Geometry: see drawing. Coordinates: mm, zero at the bounding-box minimum. A direction names the side the tool comes from. Give positions to 0.01 mm unless a question says otherwise; leave off trailing zeros. Order: outer loops, then holes, each group sorted by start corner. A loop starts at its lowest first (then second) coordinate and runs counter-clockwise, first axis right, second up. Notation, with made-up numbers: (83, 3) - (90, 3) arc R21 ccw to (90, 32) - close; hole circle Ø10 at (-36.75, 83.5). An arc over 180 degrees is marked (long way). One line per item, written item: value.
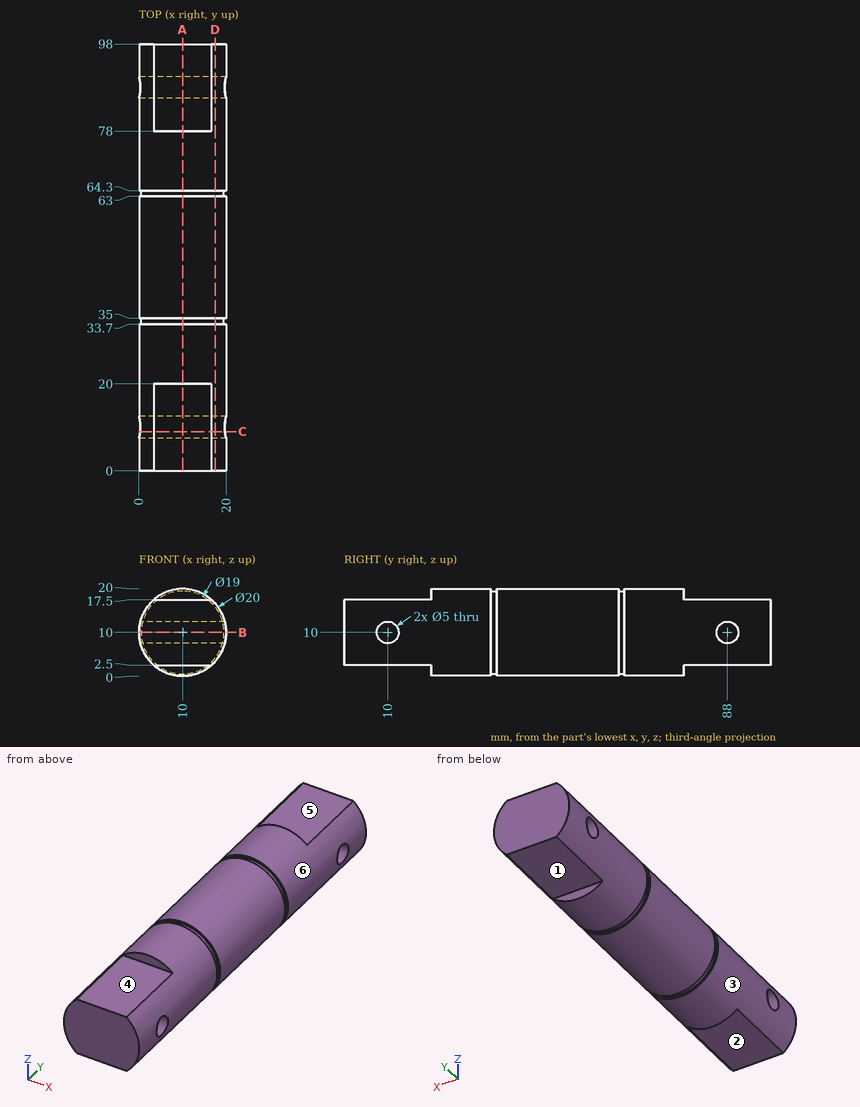
1) Section D-D, the plane x = 17.5. Return loops of the section in (y, z), then the cut area to 3 significant figures.
Answers below:
outline: (0, 3.39) - (33.7, 3.39) - (33.7, 4.17) - (35, 4.17) - (35, 3.39) - (63, 3.39) - (63, 4.17) - (64.3, 4.17) - (64.3, 3.39) - (98, 3.39) - (98, 16.61) - (64.3, 16.61) - (64.3, 15.83) - (63, 15.83) - (63, 16.61) - (35, 16.61) - (35, 15.83) - (33.7, 15.83) - (33.7, 16.61) - (0, 16.61) - close; hole circle Ø5 at (10, 10); hole circle Ø5 at (88, 10)
area: 1,250 mm^2
2) Section B-B, the plane z = 10. Return loops of the section in (x, y).
Answers below:
outline: (0, 0) - (20, 0) - (20, 7.5) - (0, 7.5) - close; (0, 12.5) - (20, 12.5) - (20, 33.7) - (19.5, 33.7) - (19.5, 35) - (20, 35) - (20, 63) - (19.5, 63) - (19.5, 64.3) - (20, 64.3) - (20, 85.5) - (0, 85.5) - (0, 64.3) - (0.5, 64.3) - (0.5, 63) - (0, 63) - (0, 35) - (0.5, 35) - (0.5, 33.7) - (0, 33.7) - close; (0, 90.5) - (20, 90.5) - (20, 98) - (0, 98) - close
3) First-contact query: pin 1 (0.8 mm diameter, centred on x = 11.5, z = 0.5, fed in from -Y); pin 2 (3 mm diameter, centred on x = 5.5, y = 29, fed in from -Z); pin 3 (0.8 mm diameter, centred on x = 7.5, z = 0.5, fed in from +Y). Flat tips, straight axial feed; report the tip coordinate or a pass-through.
Answers below:
pin 1: y = 20
pin 2: z = 0.46
pin 3: y = 78
4) Mould query, pull axis X, two halves, no side actions, for the marked faces 5 and 6. Classes: released by +X, released by -X, zero draft, split by the parting line, or undercut.
Answers below:
face 5: zero draft
face 6: split by the parting line
5) Set-up query: the marked faces 1, 2, 3 and 4. Return all of +Z, -Z, +X, -X, +Y, -Y with unobstructed straight access to the full face (end or side cutting, diameter ignored); none if empty.
Answers below:
face 1: -Z, +X, -X, +Y
face 2: -Z, +X, -X, -Y
face 3: +Y, -Y
face 4: +Z, +X, -X, -Y
6) Section C-C, the plane y = 9. Return loops of the section in (x, z).
Answers below:
outline: (0.27, 7.71) arc R10 ccw to (3.39, 2.5) - (16.61, 2.5) arc R10 ccw to (19.73, 7.71) - close; (0.27, 12.29) - (19.73, 12.29) arc R10 ccw to (16.61, 17.5) - (3.39, 17.5) arc R10 ccw to start
7) Material intervals for line 1 along Y through (x, z) = (6.75, 10); line 2 along Y through (x, z) = (5.75, 9); line 3 along Z through (x, y) = (16.75, 10.5), sorted ascending.
Answers below:
line 1: 0 to 7.5, 12.5 to 85.5, 90.5 to 98
line 2: 0 to 7.71, 12.29 to 85.71, 90.29 to 98
line 3: 2.62 to 7.55, 12.45 to 17.38
8) Section A-A, the plane x = 10. Count the separate pieces of the cut face and the enclosed holes in it, then the cut area to 3 significant figures.
Answers below:
separate pieces: 1
enclosed holes: 2
area: 1,720 mm^2
